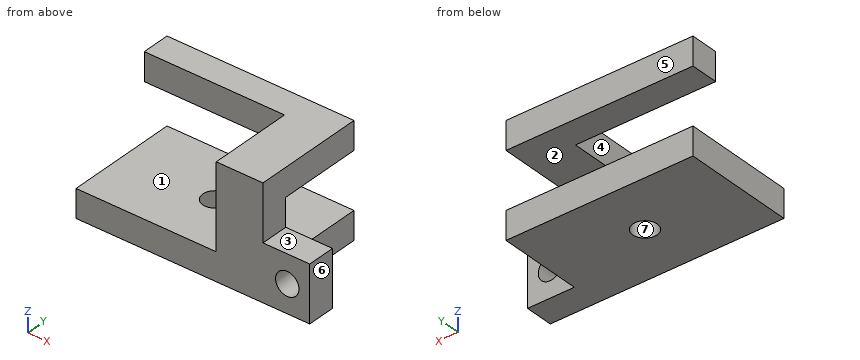
```python
from build123d import *

# Parameters (mm, degrees)
CHANNEL_PROFILE_SKETCH_W = 100
CHANNEL_PROFILE_SKETCH_H = 60
CHANNEL_PROFILE_SKETCH_R = 6.5
CHANNEL_BODY_DEPTH       = 15
LUG_1_PROFILE_SKETCH_R   = 6.266086447
PIERCED_LUG_1_DEPTH      = 15
PIERCED_LUG_2_DEPTH      = 15


with BuildPart() as part:
    # Channel Profile Sketch → Channel Body (new body)
    with BuildSketch(Plane.XY):
        Rectangle(CHANNEL_PROFILE_SKETCH_W, CHANNEL_PROFILE_SKETCH_H)
        Circle(CHANNEL_PROFILE_SKETCH_R, mode=Mode.SUBTRACT)
    extrude(amount=CHANNEL_BODY_DEPTH)

    # Lug 1 Profile Sketch → Pierced Lug 1 (add)
    with BuildSketch(Plane.XZ.offset(30)):
        Polygon((25, 0), (75, 0), (75, 30), (50, 30), (50, 60), (25, 60), align=None)
        with Locations(Location((63, 15, 0), (0, 0, 270))):
            Circle(LUG_1_PROFILE_SKETCH_R, mode=Mode.SUBTRACT)
    extrude(amount=-PIERCED_LUG_1_DEPTH)

    # Lug 2 Profile Sketch → Pierced Lug 2 (add)
    with BuildSketch(Plane.XY.offset(60)):
        Polygon((25, -30), (50, -30), (50, 30), (-50, 30), (-50, 15), (25, 15), align=None)
    extrude(amount=-PIERCED_LUG_2_DEPTH)


solid = part.part
```
CAD build for the part. Positions are in the model's coordinates, mm. Face numbers are marked on the shaded views. A direction names the side the tool comes from. Coordinates: 2 decimals unless noted, no trailing zeros. Write each loop counter-clockwise with the first axis right and the second up, starting at its lowest first coordinate (ties: lowest second). Pieces come first, ordered by that corner, then holes. Notation, with made-up numbers: (19, 30) -> (23, 30) arc R5 cw to (23, 38) -> close; hole circle Ø11 at (-17.75, -34.75). An arc over 180 degrees is marked (long way). Use CSV: the item, a comma, the result in double quotes. Start each with the question number.
Item 1: Band-saw the part on A-A, the plane y = 0. Write the cut outline in (x, z), plus the area to 3 significant figures.
Item 2: Drop flat-ended pins along their axis: P1, Ø7.5, axis at x = 63, z = 15, coming from the -Y side; P2, Ø12, axis at y = -11.5, z = 47, coming from the +X side; P3, Ø4.5, axis at x = 59, y = -21.5, coming from the +Z side; P4, Ø13.5, axis at x = 54, z = 29, coming from the +Y side. Give the stop position or say it passes through.
Item 3: Tool access for the marked faces 1, 2, 3 and 4: list every direction of +Z, -Z, +X, -X, +Y, -Y with a clear straight run to the whole face (end or side of a thin tool).
Item 4: Band-saw the part on C-C, the plane y = -13. Write the cut outline in (x, z).
Item 5: Band-saw the part on B-B, the plane x = -31.5. Write the cut outline in (y, z).
Item 6: Band-saw the part on D-D, the plane x = 0. Write the cut outline in (y, z).
Item 7: Wall check: probe 1 along Y at (x, z) = (0, 7.5); probe 2 along Z at (x, y) = (37, 3.5); probe 3 along X at (y, z) = (-3, 50). Give the ranges that are in metal, low to high.
Item 8: Two-plate mould, pull along Y, no slides. Class the marked faces 5, 6 and 7: +Y half, -Y half, draft (parallel to the pull), parting line (faces both ways), or undercut.
Response values:
1,outline,"(-50, 0) -> (-6.5, 0) -> (-6.5, 15) -> (-50, 15) -> close; (6.5, 0) -> (50, 0) -> (50, 15) -> (6.5, 15) -> close; (25, 45) -> (50, 45) -> (50, 60) -> (25, 60) -> close"
1,area,"1,680 mm2"
2,P1,"passes through"
2,P2,"stops at x = 50"
2,P3,"stops at z = 30"
2,P4,"stops at y = -15"
3,face 1,"-X, +Y"
3,face 2,"+X, -X, +Y"
3,face 3,"+Z, +X, +Y, -Y"
3,face 4,"+Z, -X, -Y"
4,outline,"(-50, 0) -> (50, 0) -> (50, 15) -> (-50, 15) -> close; (25, 45) -> (50, 45) -> (50, 60) -> (25, 60) -> close"
5,outline,"(-30, 0) -> (30, 0) -> (30, 15) -> (-30, 15) -> close; (15, 45) -> (30, 45) -> (30, 60) -> (15, 60) -> close"
6,outline,"(-30, 0) -> (-6.5, 0) -> (-6.5, 15) -> (-30, 15) -> close; (6.5, 0) -> (30, 0) -> (30, 15) -> (6.5, 15) -> close; (15, 45) -> (30, 45) -> (30, 60) -> (15, 60) -> close"
7,probe 1,"y = -30 to -6.5, 6.5 to 30"
7,probe 2,"z = 0 to 15, 45 to 60"
7,probe 3,"x = 25 to 50"
8,face 5,"+Y half"
8,face 6,"draft"
8,face 7,"undercut"
